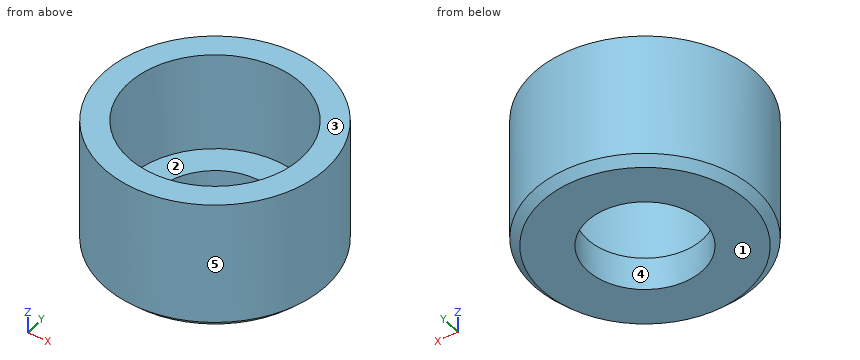
from build123d import *

# Parameters (mm, degrees)
SKETCH1_R           = 27
SKETCH1_R_2         = 14
BOSS_EXTRUDE1_DEPTH = 32
SKETCH2_R           = 21
CUT_EXTRUDE1_DEPTH  = 24
CHAMFER1_SIZE       = 2


with BuildPart() as part:
    # Sketch1 → Boss-Extrude1 (new body)
    with BuildSketch(Plane.XY):
        Circle(SKETCH1_R)
        Circle(SKETCH1_R_2, mode=Mode.SUBTRACT)
    extrude(amount=BOSS_EXTRUDE1_DEPTH)

    # Sketch2 → Cut-Extrude1 (cut)
    with BuildSketch(Plane.XY.offset(32)):
        Circle(SKETCH2_R)
    extrude(amount=-CUT_EXTRUDE1_DEPTH, mode=Mode.SUBTRACT)

    # Chamfer1
    chamfer1_edges = [part.edges().sort_by_distance(p)[0] for p in [
        (-27, 0, 0),
    ]]
    chamfer(chamfer1_edges, length=CHAMFER1_SIZE)


solid = part.part
Verification items for the finished model (mm, model axes). Face numbers are marked on the shaded views. A direction names the side the tool comes from. Give positions to 0.01 mm unless a question says otherwise; leave off trailing zeros. Loops run counter-clockwise (first coordinate to the right, second up) from the corner with the lowest first, then second, coordinate; pieces in that order, holes last. Notation, with made-up numbers: (13, 65.25) - (18, 65.25) arc R9 cw to (18, 71.25) - close; hole circle Ø10 at (50.25, 17.5). An arc over 180 degrees is marked (long way). Write each question's results on one line, items separated by ' | '.
1) Mould release check, pull along Y, two halves, no side actions. Record for the marked faces 3, 4 and 5: pulls with the +Y half, pulls with the -Y half, needs draft (parallel to the pull), parting line crosses it, or undercut.
Solution:
face 3: needs draft | face 4: undercut | face 5: parting line crosses it
2) Sectioned sample at A-A on x = 0. Record the boundary of the cut face in (y, z).
Solution:
outline: (-27, 2) - (-25, 0) - (-14, 0) - (-14, 8) - (-21, 8) - (-21, 32) - (-27, 32) - close; (14, 0) - (25, 0) - (27, 2) - (27, 32) - (21, 32) - (21, 8) - (14, 8) - close
3) Tool access check on the marked faces 1 and 2. Record the directions out of +Z, -Z, +X, -X, +Y, -Y that give a thin tool (end or side, any length) a straight path to the whole face; none if there is none.
Solution:
face 1: -Z, +X, -X, +Y, -Y | face 2: +Z
4) Depth check by flat-ended pin: P1, Ø1.5, axis at x = 16, y = -12, coming from the +Z side; P2, Ø12, axis at x = -15.5, y = 16, coming from the -Z side; P3, Ø2, axis at x = 21.5, z = 7, coming from the +Y side; P4, Ø8, axis at x = -21, z = 15.5, coming from the +Y side. Enter the tip coordinate at first touch or a pass-through.
Solution:
P1: z = 8 | P2: z = 0 | P3: y = 17.57 | P4: y = 20.98
5) Sectioned sample at C-C on z = 26. Record the boundary of the cut face in (x, y).
Solution:
outline: circle Ø54 at (0, 0); hole circle Ø42 at (0, 0)
6) Material ranges on L1, parallel to Y at x = 0, z = 24; L2, parallel to Y at x = 0, z = 4; L3, parallel to Z at x = 13.5, y = -7.5, recorded low to high. Write a range as from..to.
Solution:
L1: -27..-21, 21..27 | L2: -27..-14, 14..27 | L3: 0..8
